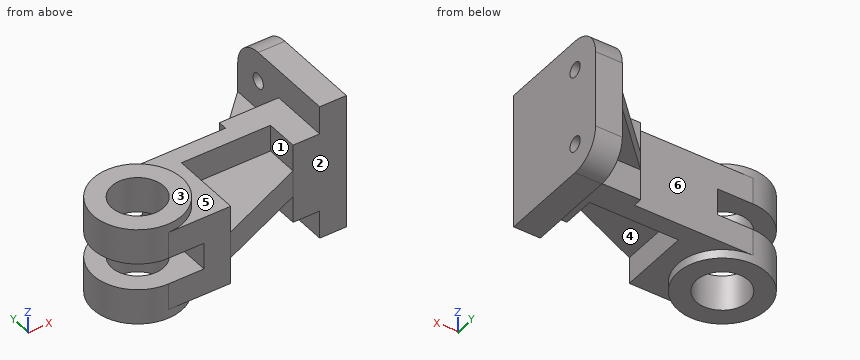
```python
from build123d import *

# Parameters (mm, degrees)
HUB_PROFILE_R                = 30
HUB_PROFILE_R_2              = 17.5
BEARING_HUB_60_BORE_35_DEPTH = 33
SUPPORT_ARM_DEPTH            = 27
HUB_RIB_18_REACH             = 131.557
HUB_RIB_SKETCH_WALL_W        = 326.505005478
HUB_RIB_SKETCH_WALL_H        = 18
MOUNTING_PLATE_PROFILE_R     = 5
MOUNTING_PLATE_DEPTH         = 18
PLATE_RIB_12_REACH           = 166.122
PLATE_RIB_SKETCH_WALL_W      = 386.812354318
PLATE_RIB_SKETCH_WALL_H      = 12
FORK_SLOT_PROFILE_W          = 57.638691925
FORK_SLOT_PROFILE_H          = 18
FORK_SLOT_24X18_DEPTH        = 158.353106102


with BuildPart() as part:
    # Hub Profile → Bearing Hub Ø60 Bore Ø35 (new, symmetric)
    with BuildSketch(Plane.XY):
        Circle(HUB_PROFILE_R)
        Circle(HUB_PROFILE_R_2, mode=Mode.SUBTRACT)
    extrude(amount=BEARING_HUB_60_BORE_35_DEPTH, both=True)

    # Support Arm Profile → Support Arm (add, symmetric)
    with BuildSketch(Plane.XY):
        with BuildLine():
            Line((0, 30), (45.688517283, 30))
            Line((45.688517283, 30), (80, 30))
            Line((80, 30), (80, 36))
            Line((80, 36), (120, 36))
            Line((120, 36), (120, -4))
            Line((120, -4), (102, -4))
            Line((102, -4), (102, 18))
            Line((102, 18), (42, 18))
            Line((42, 18), (42, -30))
            Line((42, -30), (0, -30))
            ThreePointArc((0, -30), (30, 0), (0, 30))
        make_face()
    extrude(amount=SUPPORT_ARM_DEPTH, both=True)

    # Hub Rib Sketch wall → Hub Rib 18 (add, up to next)
    with BuildSketch(Plane(origin=(72, -17, 0), x_dir=(0.91755562531, 0.397607437634, 0), z_dir=(-0.397607437634, 0.91755562531, 0)), mode=Mode.PRIVATE) as hub_rib_18_sk1:
        Rectangle(HUB_RIB_SKETCH_WALL_W, HUB_RIB_SKETCH_WALL_H)
    hub_rib_18_tool1 = extrude(hub_rib_18_sk1.sketch, amount=HUB_RIB_18_REACH, mode=Mode.PRIVATE) - part.part
    add(hub_rib_18_tool1.solids().sort_by_distance((72, -17, 0))[0])

    # Mounting Plate Profile → Mounting Plate (add)
    with BuildSketch(Plane(origin=(120, 0, 0), x_dir=(0, 0, -1), z_dir=(1, 0, 0))):
        with BuildLine():
            Line((-46, -4), (46, -4))
            Line((46, -4), (46, 56))
            ThreePointArc((46, 56), (40.142135624, 70.142135624), (26, 76))
            Line((26, 76), (-26, 76))
            ThreePointArc((-26, 76), (-40.142135624, 70.142135624), (-46, 56))
            Line((-46, 56), (-46, -4))
        make_face()
        with Locations((-26, 56)):
            Circle(MOUNTING_PLATE_PROFILE_R, mode=Mode.SUBTRACT)
        with Locations((26, 56)):
            Circle(MOUNTING_PLATE_PROFILE_R, mode=Mode.SUBTRACT)
    extrude(amount=MOUNTING_PLATE_DEPTH)

    # Plate Rib Sketch wall → Plate Rib 12 (add, up to next)
    with BuildSketch(Plane(origin=(100, 56, 0), x_dir=(0.707106781187, 0.707106781187, 0), z_dir=(-0.707106781187, 0.707106781187, 0)), mode=Mode.PRIVATE) as plate_rib_12_sk1:
        Rectangle(PLATE_RIB_SKETCH_WALL_W, PLATE_RIB_SKETCH_WALL_H)
    plate_rib_12_tool1 = extrude(plate_rib_12_sk1.sketch, amount=-PLATE_RIB_12_REACH, mode=Mode.PRIVATE) - part.part
    add(plate_rib_12_tool1.solids().sort_by_distance((100, 56, 0))[0])

    # Fork Slot Profile → Fork Slot 24x18 (cut, through all)
    with BuildSketch(Plane(origin=(0, 30, 0), x_dir=(1, 0, 0), z_dir=(0, 1, 0))):
        with Locations((-4.819345963, 0)):
            Rectangle(FORK_SLOT_PROFILE_W, FORK_SLOT_PROFILE_H)
    extrude(amount=-FORK_SLOT_24X18_DEPTH, mode=Mode.SUBTRACT)


solid = part.part
```
Can you work these out from the model? Positions are in its coordinate system, mm. Face numbers are marked on the shaded views. A direction names the side the tool comes from. Give positions to 0.01 mm unless a question says otherwise; leave off trailing zeros. Order: outer loops, then holes, each group sorted by start corner. A loop starts at its lowest first (then second) coordinate and runs counter-clockwise, first axis right, second up. Notation, with made-up numbers: M 21,63.5 L 34,63.5 A10 ccw 34,74.5 Z; hole C 0.25,44.25 d1. An arc over 180 degrees is marked long. Write item = value, one per line. Start each with the question number.
Q1. Suppose I cut it at B-B (x = 104.5). Write out the boundary of the cut face in (y, z), plus the area to 3 significant figures.
Q2. Suppose I cut it at D-D (z = 35). Write out the boundary of the cut face in (x, y), plus the area to 3 significant figures.
Q3. Suppose I cut it at C-C (y = 45). Write out the boundary of the cut face in (x, z), plus the area to 3 significant figures.
Q4. Will these pins go through, and if not, where does the flat tip stop? pin 1 Ø6 at (y, z) = (-12, -28) entering from -X; pin 2 Ø20 at (x, z) = (61, 16) entering from -Y; pin 3 Ø12 at (y, z) = (30.5, -10.5) entering from -X; pin 4 Ø16 at (x, y) = (1, -5) entering from -Z.
Q5. I need wall thicknesses on probe 1 along X at (y, z) = (0, 17.75); probe 2 along Y at (x, z) = (125, 26); probe 3 along Y at (x, z) = (0, -27.25). Which ranges of each line are inside material? Lowest first, please. Write a range as [from, to].
Q6. Suppose I cut it at A-A (y = 0). Count the separate pieces of the cut face and the enclosed holes in it, plus the area to 3 significant figures.
Q7. For the marked faces 1, 2, 3 and 4, which set-ups out of +Z, -Z, +X, -X, +Y, -Y let a thin tool reach every point of the face, with its end or its side?
Q8. We'd pull the mould along X, two halves only. Please class the marked faces 5 and 6: pulls with the +X half, pulls with the -X half, needs draft (parallel to the pull), parting line crosses it, or undercut.
Check result:
q1.outline = M -4,-27 L 36,-27 L 36,-6 L 60.5,-6 L 60.5,6 L 36,6 L 36,27 L -4,27 Z
q1.area = 2,450 mm2
q2.outline = M 120,-4 L 138,-4 L 138,73.86 L 120,73.86 Z
q2.area = 1,400 mm2
q3.outline = M 89,-6 L 120,-6 L 120,-46 L 138,-46 L 138,46 L 120,46 L 120,6 L 89,6 Z
q3.area = 2,030 mm2
q4.pin_1 = -28.62
q4.pin_2 = -24.86
q4.pin_3 = -17.31
q4.pin_4 = through
q5.probe_1 = [-30, -17.5], [17.5, 42], [102, 138]
q5.probe_2 = [-4, 51], [61, 76]
q5.probe_3 = [-30, -17.5], [17.5, 30]
q6.separate_pieces = 3
q6.enclosed_holes = 0
q6.area = 5,660 mm2
q7.face_1 = +Z, -Y
q7.face_2 = +Z, -Z, +X, -Y
q7.face_3 = +Z, -X, +Y, -Y
q7.face_4 = -Z, -Y
q8.face_5 = undercut
q8.face_6 = needs draft
